```python
from build123d import *

# Parameters (mm, degrees)
SKETCH_1_W          = 40
SKETCH_1_H          = 60
EXTRUDE_1_DEPTH     = 10
SKETCH_2_W          = 38
SKETCH_2_H          = 58
EXTRUDE_2_DEPTH     = 2
SKETCH_3_W          = 40
SKETCH_3_H          = 60
EXTRUDE_3_DEPTH     = 3
SKETCH_4_R          = 20
EXTRUDE_4_DEPTH     = 10
EXTRUDE_5_DEPTH     = 10
SKETCH_6_R          = 1.65
CUT_EXTRUDE_1_DEPTH = 20
EXTRUDE_6_DEPTH     = 30
SKETCH_8_R          = 15
EXTRUDE_7_DEPTH     = 5
SKETCH_9_R          = 10
EXTRUDE_8_DEPTH     = 10
SKETCH_10_W         = 25
SKETCH_10_H         = 18.68197258
EXTRUDE_9_DEPTH     = 10
SKETCH_11_R         = 2.2
CUT_EXTRUDE_2_DEPTH = 10
SKETCH_12_W         = 20
SKETCH_12_H         = 60
EXTRUDE_10_DEPTH    = 34
SKETCH_13_R         = 2.2
CUT_EXTRUDE_3_DEPTH = 35


with BuildPart() as part:
    # 草图1 → 凸台-拉伸1 (new body)
    with BuildSketch(Plane.XY):
        Rectangle(SKETCH_1_W, SKETCH_1_H)
    extrude(amount=EXTRUDE_1_DEPTH)

    # 草图2 → 凸台-拉伸2 (add)
    with BuildSketch(Plane.XY.offset(10)):
        Rectangle(SKETCH_2_W, SKETCH_2_H)
    extrude(amount=EXTRUDE_2_DEPTH)

    # 草图3 → 凸台-拉伸3 (add)
    with BuildSketch(Plane.XY.offset(12)):
        Rectangle(SKETCH_3_W, SKETCH_3_H)
    extrude(amount=EXTRUDE_3_DEPTH)

    # 草图4 → 凸台-拉伸4 (add)
    with BuildSketch(Plane.XY.offset(15)):
        Circle(SKETCH_4_R)
    extrude(amount=EXTRUDE_4_DEPTH)

    # 草图5 → 凸台-拉伸5 (add)
    with BuildSketch(Plane.XY.offset(25)):
        with BuildLine():
            Line((9.142135624, -14.142135624), (-9.142135624, -14.142135624))
            ThreePointArc((-9.142135624, -14.142135624), (-12.67766953, -12.67766953), (-14.142135624, -9.142135624))
            Line((-14.142135624, -9.142135624), (-14.142135624, 9.142135624))
            ThreePointArc((-14.142135624, 9.142135624), (-12.67766953, 12.67766953), (-9.142135624, 14.142135624))
            Line((-9.142135624, 14.142135624), (9.142135624, 14.142135624))
            ThreePointArc((9.142135624, 14.142135624), (12.67766953, 12.67766953), (14.142135624, 9.142135624))
            Line((14.142135624, 9.142135624), (14.142135624, -9.142135624))
            ThreePointArc((14.142135624, -9.142135624), (12.67766953, -12.67766953), (9.142135624, -14.142135624))
        make_face()
    extrude(amount=EXTRUDE_5_DEPTH)

    # 草图6 → 切除-拉伸1 (cut)
    with BuildSketch(Plane(origin=(0, 0, 0), x_dir=(-1, 0, 0), z_dir=(0, 0, -1))):
        with Locations((17, 27)):
            Circle(SKETCH_6_R)
        with Locations((17, -27)):
            Circle(SKETCH_6_R)
        with Locations((-17, -27)):
            Circle(SKETCH_6_R)
        with Locations((-17, 27)):
            Circle(SKETCH_6_R)
    extrude(amount=-CUT_EXTRUDE_1_DEPTH, mode=Mode.SUBTRACT)

    # 草图7 → 凸台-拉伸6 (add)
    with BuildSketch(Plane.XY.offset(35)):
        Polygon((20, -20), (20, 20), (-20, 20), (-20, 10), (-30, 10), (-30, -20), align=None)
    extrude(amount=EXTRUDE_6_DEPTH)

    # 草图8 → 凸台-拉伸7 (add)
    with BuildSketch(Plane.XY.offset(65)):
        Circle(SKETCH_8_R)
    extrude(amount=EXTRUDE_7_DEPTH)

    # 草图9 → 凸台-拉伸8 (add)
    with BuildSketch(Plane.XY.offset(70)):
        Circle(SKETCH_9_R)
    extrude(amount=EXTRUDE_8_DEPTH)

    # 草图10 → 凸台-拉伸9 (add)
    with BuildSketch(Plane(origin=(20, 0, 0), x_dir=(0, 0, -1), z_dir=(1, 0, 0))):
        with Locations((-47.5, 29.34098629)):
            Rectangle(SKETCH_10_W, SKETCH_10_H)
        with Locations((-47.5, -29.34098629)):
            Rectangle(SKETCH_10_W, SKETCH_10_H)
    extrude(amount=-EXTRUDE_9_DEPTH)

    # 草图11 → 切除-拉伸2 (cut)
    with BuildSketch(Plane.ZY.offset(-10)):
        with Locations((55, 33.68197258)):
            Circle(SKETCH_11_R)
        with Locations((40, 33.68197258)):
            Circle(SKETCH_11_R)
        with Locations((40, -33.68197258)):
            Circle(SKETCH_11_R)
        with Locations((55, -33.68197258)):
            Circle(SKETCH_11_R)
    extrude(amount=-CUT_EXTRUDE_2_DEPTH, mode=Mode.SUBTRACT)

    # 草图12 → 凸台-拉伸10 (add)
    with BuildSketch(Plane.XY.offset(80)):
        with Locations((0, 10)):
            Rectangle(SKETCH_12_W, SKETCH_12_H)
    extrude(amount=EXTRUDE_10_DEPTH)

    # 草图13 → 切除-拉伸3 (cut)
    with BuildSketch(Plane.ZY.offset(10)):
        with Locations(Location((108, 34, 0), (0, 0, 270))):
            Circle(SKETCH_13_R)
        with Locations(Location((86, 34, 0), (0, 0, 270))):
            Circle(SKETCH_13_R)
        with Locations(Location((108, -14, 0), (0, 0, 270))):
            Circle(SKETCH_13_R)
        with Locations(Location((86, -14, 0), (0, 0, 270))):
            Circle(SKETCH_13_R)
    extrude(amount=-CUT_EXTRUDE_3_DEPTH, mode=Mode.SUBTRACT)


solid = part.part
```
Verification items for the finished model (mm, model axes). A direction names the side the tool comes from. Round coordinates to 2 decimals unless told otherwise and drop trailing zeros. Write each loop counter-clockwise with the first axis right and the second up, starting at its lowest first coordinate (ties: lowest second). Pieces come first, ordered by that corner, then holes. Notation, with made-up numbers: (-18.75, 60) - (-5.75, 60) arc R21 cw to (-5.75, 67) - close; hole circle Ø1 at (86, 1.5). An arc over 180 degrees is marked (long way). Answer as a JSON object with one key per item and string values. Group by question number.
Q1. Thickness scan on line 1 (Z direction, x = 0, y = 34); line 2 (Z direction, x = 7.5, y = 16); line 3 (Z direction, x = -4.25, y = -14). Record the ranges inside material, lowest first.
Q2. Section check A-A, the plane z = 108. Enter the section's corners in (x, y), plus the area to 3 significant figures.
Q3. Section check D-D, the plane x = -5.5. Give the number of separate pieces and of enclosed holes in the cut face, plus the area to 3 significant figures.
Q4. Section check C-C, the plane z = 45. Enter the section's corners in (x, y).
Q5. Mould release check, pull along Y, two halves, no side actions. Record for faces 5 (the flat face through (0, 40, 97)), 6 (the flat face through (15, -38.682, 48)), 7 (the flat face through (14.142, 0, 30)), 8 (the cylindrical face through (14.93, 35.17, 53.38)): released by +Y, released by -Y, zero draft, split by the parting line, or undercut.
Q6. Go/stop test with flat-tipped pins: pin 1 Ø4 at (x, y) = (17, -27) entering from +Z; pin 2 Ø8 at (x, z) = (-22, 35.5) entering from -Y; pin 3 Ø1 at (x, z) = (8, 11) entering from -Y; pin 4 Ø2.5 at (y, z) = (33.68, 55) entering from +X. Record where each tip stops, or that it passes through.
Q7. Tool access check on faces 1 (the flat face through (0, 22, 15)), 2 (the flat face through (15, 29, 60)), 3 (the flat face through (10, -29, 48)), 4 (the flat face through (0, -20, 97)). Record the directions out of +Z, -Z, +X, -X, +Y, -Y that give a thin tool (end or side, any length) a straight path to the whole face; none if there is none.
Q8. Section check B-B, the plane x = -17. Enter the section's corners in (y, z), plus the area to 3 significant figures.
Found:
{
 "1": {"line 1": "z = 80 to 83.8, 88.2 to 105.8, 110.2 to 114", "line 2": "z = 0 to 25, 35 to 65, 80 to 114", "line 3": "z = 0 to 70, 80 to 83.8, 88.2 to 105.8, 110.2 to 114"},
 "2": {"outline": "(-10, -20) - (10, -20) - (10, -16.2) - (-10, -16.2) - close; (-10, -11.8) - (10, -11.8) - (10, 31.8) - (-10, 31.8) - close; (-10, 36.2) - (10, 36.2) - (10, 40) - (-10, 40) - close", "area": "1,020 mm^2"},
 "3": {"separate pieces": "1", "enclosed holes": "4", "area": "5,050 mm^2"},
 "4": {"outline": "(-30, -20) - (10, -20) - (10, -38.68) - (20, -38.68) - (20, 38.68) - (10, 38.68) - (10, 20) - (-20, 20) - (-20, 10) - (-30, 10) - close"},
 "5": {"face 5": "released by +Y", "face 6": "released by -Y", "face 7": "zero draft", "face 8": "undercut"},
 "6": {"pin 1": "stops at z = 60", "pin 2": "stops at y = -20", "pin 3": "stops at y = -29", "pin 4": "passes through"},
 "7": {"face 1": "+Y", "face 2": "+Z, +X, -X, +Y", "face 3": "+Z, -X, -Y", "face 4": "+Z, +X, -X, -Y"},
 "8": {"outline": "(-30, 0) - (-28.65, 0) - (-28.65, 15) - (-30, 15) - (-30, 12) - (-29, 12) - (-29, 10) - (-30, 10) - close; (-25.35, 0) - (25.35, 0) - (25.35, 15) - (10.54, 15) - (10.54, 25) - (-10.54, 25) - (-10.54, 15) - (-25.35, 15) - close; (-20, 35) - (20, 35) - (20, 65) - (-20, 65) - close; (28.65, 0) - (30, 0) - (30, 10) - (29, 10) - (29, 12) - (30, 12) - (30, 15) - (28.65, 15) - close", "area": "2,210 mm^2"}
}
